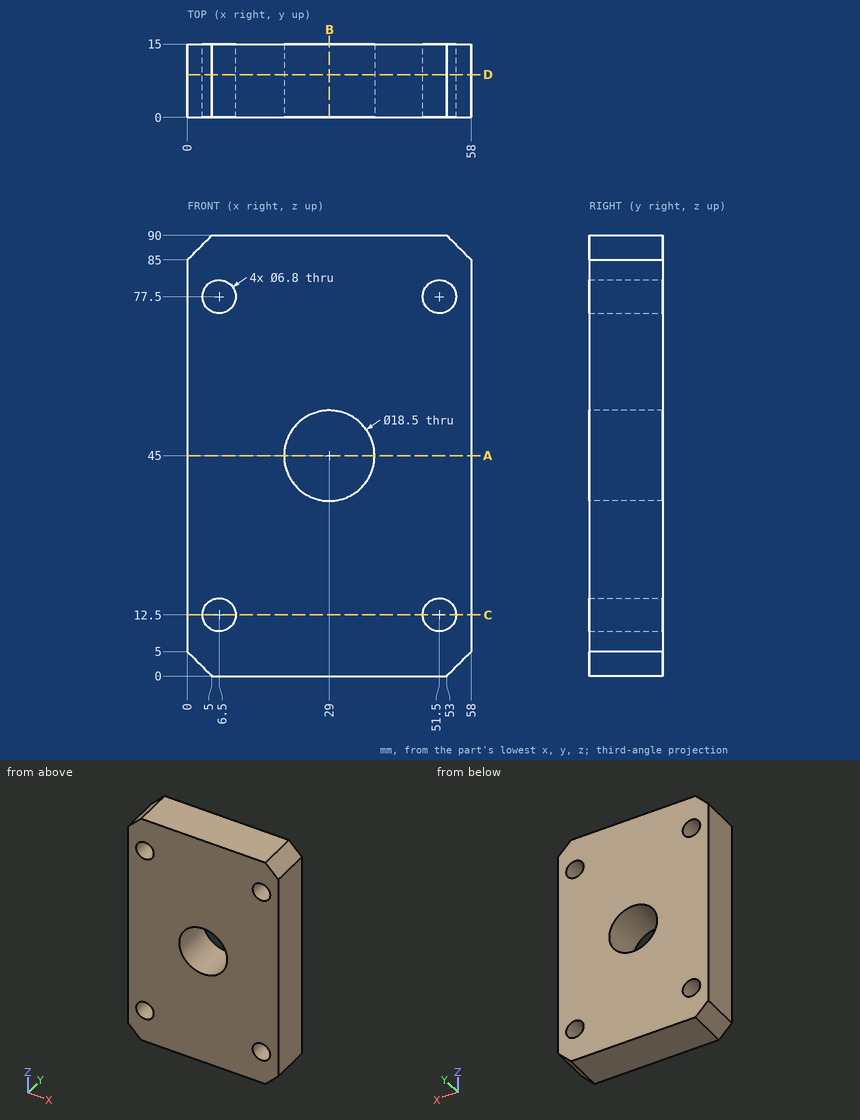
Can you work these out from the drawing? Everything is in mm from the part's minimum corner. Round coordinates to 2 decimals unless told otherwise and drop trailing zeros. Write each loop counter-clockwise with the first axis right and the second up, starting at its lowest first coordinate (ties: lowest second). Pieces come first, ordered by that corner, then holes.
1. Suppose I cut it at B-B (x = 29). List the corners of the cut face in (y, z) for me, and give its area (3 significant figures).
2. Suppose I cut it at A-A (z = 45). List the corners of the cut face in (x, y) for me.
3. Suppose I cut it at D-D (y = 8.75). List the corners of the cut face in (x, z) for me.
4. Will this pin go through, and if not, where does the flat tip stop? pin 1 Ø2 at (x, y) = (35, 13) entering from -Z.
5. I need wall thicknesses on L1, parallel to Z at x = 51.5, y = 7.25; L2, parallel to X at y = 5, z = 10; L3, parallel to Z at x = 5.5, y = 6.5. Which ranges of each line are inside material? Lowest first, please.
6. Suppose I cut it at C-C (z = 12.5). List the corners of the cut face in (x, y) for me, and give its area (3 significant figures).
Answer sheet:
1. outline: (0, 0) - (15, 0) - (15, 35.75) - (0, 35.75) - close; (0, 54.25) - (15, 54.25) - (15, 90) - (0, 90) - close
1. area: 1,070 mm2
2. outline: (0, 0) - (19.75, 0) - (19.75, 15) - (0, 15) - close; (38.25, 0) - (58, 0) - (58, 15) - (38.25, 15) - close
3. outline: (0, 5) - (5, 0) - (53, 0) - (58, 5) - (58, 85) - (53, 90) - (5, 90) - (0, 85) - close; hole circle Ø6.8 at (6.5, 12.5); hole circle Ø6.8 at (6.5, 77.5); hole circle Ø18.5 at (29, 45); hole circle Ø6.8 at (51.5, 12.5); hole circle Ø6.8 at (51.5, 77.5)
4. pin 1: stops at z = 0
5. L1: z = 0 to 9.1, 15.9 to 74.1, 80.9 to 90
5. L2: x = 0 to 4.2, 8.8 to 49.2, 53.8 to 58
5. L3: z = 0 to 9.25, 15.75 to 74.25, 80.75 to 90
6. outline: (0, 0) - (3.1, 0) - (3.1, 15) - (0, 15) - close; (9.9, 0) - (48.1, 0) - (48.1, 15) - (9.9, 15) - close; (54.9, 0) - (58, 0) - (58, 15) - (54.9, 15) - close
6. area: 666 mm2
